CAD build for the part. Positions are in the model's coordinates, mm. A direction names the side the tool comes from. Round coordinates to 2 decimals unless told otherwise and drop trailing zeros. Use one line per item in the form item = value. Start each with the question number.
Item 1: Pin check, flat tips, straight feed: pin 1 (8 mm diameter, centred on x = -5.5, y = 2.5, fed in from -Z); pin 2 (9 mm diameter, centred on x = -4.5, y = 0, fed in from -Z); pin 3 (3.5 mm diameter, centred on y = 17.5, z = 5, fed in from +X); pin 4 (5 mm diameter, centred on x = 165.5, y = 0, fed in from +Z). Stop position of each tip, or through.
Item 2: Drill centre lines: L1, parallel to Y at x = -188.5, z = 5; L2, parallel to Y at x = -89.5, z = 8.5; L3, parallel to Y at x = -4.5, z = 2.8. Where is each one in solid material? Low to high.
Item 3: Tool access for faces 1 (the cylindrical face through (170.495, 0.22, 2.81)), 2 (the flat face through (-198, 0, 5)): list every direction of +Z, -Z, +X, -X, +Y, -Y with a clear straight run to the whole face (end or side of a thin tool).
Item 4: Pull direction X, two halves, no side cores. Call faces 3 (the flat face through (198, 0, 5)), 4 (the cylindrical face through (75.881, -1.915, 2.81)), 5 (the flat face through (-3, 7, 10)): +X half, -X half, draft (parallel to the pull), parting line (faces both ways), or undercut.
from build123d import *

# Parameters (mm, degrees)
SKETCH1_W                                            = 396
SKETCH1_H                                            = 60
BOSS_EXTRUDE1_DEPTH                                  = 10
HOLE_SIZE_PER_SOCKET_HEAD_CAP_SCREW_TYPE_D           = 5.5
HOLE_SIZE_PER_SOCKET_HEAD_CAP_SCREW_TYPE_CBORE_D     = 10
HOLE_SIZE_PER_SOCKET_HEAD_CAP_SCREW_TYPE_CBORE_DEPTH = 5.7
M5_TAPPED_HOLE1_AT_2_COUNT                           = 2
M5_TAPPED_HOLE1_AT_2_PITCH                           = 35


with BuildPart() as part:
    # Sketch1 → Boss-Extrude1 (new body)
    with BuildSketch(Plane.XY):
        Rectangle(SKETCH1_W, SKETCH1_H)
    extrude(amount=BOSS_EXTRUDE1_DEPTH)

    # Hole size per socket head cap screw type 1 (through all)
    with Locations(Plane(origin=(0, 0, 0), x_dir=(-1, 0, 0), z_dir=(0, 0, -1))):
        with Locations((89.5, 0), (4.5, 0), (-80.5, 0), (-165.5, 0)):
            CounterBoreHole(HOLE_SIZE_PER_SOCKET_HEAD_CAP_SCREW_TYPE_D / 2, HOLE_SIZE_PER_SOCKET_HEAD_CAP_SCREW_TYPE_CBORE_D / 2, HOLE_SIZE_PER_SOCKET_HEAD_CAP_SCREW_TYPE_CBORE_DEPTH)

    # Sketch4 → M5 Tapped Hole1 (revolve, cut)
    with BuildSketch(Plane(origin=(-198, 17.5, 5), x_dir=(0, 0, 1), z_dir=(0, 1, 0))):
        Polygon((0, 0), (0, 13.6618073), (2.1, 12.4), (2.1, 0), align=None)
    m5_tapped_hole1 = revolve(axis=Axis((-204.35, 17.5, 5), (1, 0, 0)), mode=Mode.SUBTRACT)

    # M5 Tapped Hole1 at 2: M5 Tapped Hole1 ×2
    with Locations(*[(0, -i * M5_TAPPED_HOLE1_AT_2_PITCH, 0) for i in range(1, M5_TAPPED_HOLE1_AT_2_COUNT)]):
        add(m5_tapped_hole1, mode=Mode.SUBTRACT)

    # Mirror1: M5 Tapped Hole1 across plane
    add(m5_tapped_hole1.mirror(Plane(origin=(0, 0, 0), x_dir=(0, 0, 1), z_dir=(1, 0, 0))), mode=Mode.SUBTRACT)

    # Mirror1 copy 1 sketch → Mirror1 copy 1 (revolve, cut)
    with BuildSketch(Plane(origin=(198, -17.5, 5), x_dir=(0, 0, 1), z_dir=(0, 1, 0))):
        Polygon((0, 0), (0, -13.6618073), (2.1, -12.4), (2.1, 0), align=None)
    revolve(axis=Axis((204.35, -17.5, 5), (1, 0, 0)), mode=Mode.SUBTRACT)


solid = part.part
Determined:
q1.pin_1 = 0
q1.pin_2 = 5.7
q1.pin_3 = 185.39
q1.pin_4 = through
q2.L1 = -30 to -19.6, -15.4 to 15.4, 19.6 to 30
q2.L2 = -30 to -2.75, 2.75 to 30
q2.L3 = -30 to -5, 5 to 30
q3.face_1 = -Z
q3.face_2 = +Z, -Z, -X, +Y, -Y
q4.face_3 = +X half
q4.face_4 = undercut
q4.face_5 = draft
